Input: part model. Units: mm. Frame: model coordinates. A direction names the side the tool comes from. Give positions to 0.01 mm unless a question says otherwise; leave off trailing zeros. Loops run counter-clockwise (first coordinate to the right, second up) from the corner with the lowest first, then second, coordinate; pieces in that order, holes last. Notation, with made-up numbers: M 44,-30 L 80,-30 A21 cw 80,2 Z; hole C 64.5,43 d7. An arc over 180 degrees is marked long. Answer as a JSON object with one key per item and string values. Group by question number.
1) Section query B-B on x = 0. Return loops of the section in (y, z), plus the area to 3 significant figures.
2) Access query for faces 1 (the cylindrical face through (0, -22, -5)), 2 (the cylindrical face through (0, -2, -10)), 3 (the flat face through (3, -17, 3)). Directions: +Z, -Z, +X, -X, +Y, -Y. A direction counts if a zero-diameter tool reaches every point of the face in a straight line with its end or side. Return the directions, or none.
3) Section query A-A on z = 0. Return loops of the section in (x, y), plus the area to 3 significant figures.
4) Section query C-C on y = -17.5. Return loops of the section in (x, z), plus the area to 3 significant figures.
5) Ray query, L1, parallel to Y at x = -8, z = -5; L2, parallel to Y at x = 4, z = 4.5; L3, parallel to X at y = -11.5, z = 6. Return the intervals inside material, ascending.
6) Section query D-D on y = -14. Return loops of the section in (x, z), plus the area to 3 significant figures.
7) Draft query along Y for faces 4 (the flat face through (-8, -3, 1)), 5 (the flat face through (0, 0, 0)), 6 (the cylindrical face through (3.905, -18.014, -0.867)). Return one class per face: +Y half, -Y half, draft (parallel to the pull), parting line (faces both ways), or undercut.
8) First-contact query: P1, Ø12, axis at y = -22, z = -7, coming from the -X side; P2, Ø2, axis at y = -5, z = -4.5, coming from the -X side; P3, Ø2, axis at x = 6.5, y = -10, coming from the -Z side. Flat tips, straight axial feed; report the tip coordinate or a pass-through.
from build123d import *

# Parameters (mm, degrees)
CHAMFER1_SIZE = 0.5


with BuildPart() as part:
    # Sketch1 → Revolve1 (revolve)
    with BuildSketch(Plane(origin=(0, 0, 0), x_dir=(0, 0, -1), z_dir=(1, 0, 0)), mode=Mode.PRIVATE) as revolve1_sk:
        Polygon((0, 0), (10, 0), (10, -3), (7.5, -3), (7.5, -17), (4, -17), (4, -19), (5, -19), (5, -25), (0, -25), align=None)
    revolve(revolve1_sk.sketch.rotate(Axis((0, 0, 0), (0, -1, 0)), 180), axis=Axis((0, 0, 0), (0, -1, 0)))

    # Chamfer1
    chamfer1_edges = [part.edges().sort_by_distance(p)[0] for p in [
        (0, -17, -7.5),
        (0, -3, -10),
        (0, 0, -10),
        (0, -25, -5),
    ]]
    chamfer(chamfer1_edges, length=CHAMFER1_SIZE)


solid = part.part
Output:
{
 "1": {"outline": "M -25,-4.5 L -24.5,-5 L -19,-5 L -19,-4 L -17,-4 L -17,-7 L -16.5,-7.5 L -3,-7.5 L -3,-9.5 L -2.5,-10 L -0.5,-10 L 0,-9.5 L 0,9.5 L -0.5,10 L -2.5,10 L -3,9.5 L -3,7.5 L -16.5,7.5 L -17,7 L -17,4 L -19,4 L -19,5 L -24.5,5 L -25,4.5 Z", "area": "345 mm^2"},
 "2": {"face 1": "-Y", "face 2": "+Y, -Y", "face 3": "none"},
 "3": {"outline": "M -10,-2.5 L -9.5,-3 L -7.5,-3 L -7.5,-16.5 L -7,-17 L -4,-17 L -4,-19 L -5,-19 L -5,-24.5 L -4.5,-25 L 4.5,-25 L 5,-24.5 L 5,-19 L 4,-19 L 4,-17 L 7,-17 L 7.5,-16.5 L 7.5,-3 L 9.5,-3 L 10,-2.5 L 10,-0.5 L 9.5,0 L -9.5,0 L -10,-0.5 Z", "area": "345 mm^2"},
 "4": {"outline": "C 0,0 d8", "area": "50.3 mm^2"},
 "5": {"L1": "y = -3 to 0", "L2": "y = -17 to 0", "L3": "x = -4.5 to 4.5"},
 "6": {"outline": "C 0,0 d15", "area": "177 mm^2"},
 "7": {"face 4": "-Y half", "face 5": "+Y half", "face 6": "undercut"},
 "8": {"P1": "stops at x = -5.98", "P2": "stops at x = -6.63", "P3": "stops at z = -5.1"}
}
